Read the model definition and answer for the solid it produces. Units are mm, in the model's axes. A direction names the side the tool comes from. Coordinates: 2 decimals unless noted, no trailing zeros. Loops run counter-clockwise (first coordinate to the right, second up) from the corner with the lowest first, then second, coordinate; pieces in that order, holes last. Notation, with made-up numbers: (52, 28) - (79, 28) arc R15 cw to (79, 42) - close; hole circle Ø9 at (69.5, 36.5). An arc over 180 degrees is marked (long way). One line per item, written item: value. Start each with the question number.
from build123d import *

# Parameters (mm, degrees)
SKETCH_1_R          = 5.25
EXTRUDE_1_DEPTH     = 10
EXTRUDE_2_DEPTH     = 30
SKETCH_3_R          = 10
CUT_EXTRUDE_1_DEPTH = 134
FILLET_1_R          = 5


with BuildPart() as part:
    # 草图1 → 凸台-拉伸1 (new body)
    with BuildSketch(Plane.XY):
        with BuildLine():
            Line((-120, -130), (120, -130))
            ThreePointArc((120, -130), (127.071067812, -127.071067812), (130, -120))
            Line((130, -120), (130, 120))
            ThreePointArc((130, 120), (127.071067812, 127.071067812), (120, 130))
            Line((120, 130), (-120, 130))
            ThreePointArc((-120, 130), (-127.071067812, 127.071067812), (-130, 120))
            Line((-130, 120), (-130, -120))
            ThreePointArc((-130, -120), (-127.071067812, -127.071067812), (-120, -130))
        make_face()
        with Locations((-115, 115)):
            Circle(SKETCH_1_R, mode=Mode.SUBTRACT)
        with Locations((115, 115)):
            Circle(SKETCH_1_R, mode=Mode.SUBTRACT)
        with Locations((115, -115)):
            Circle(SKETCH_1_R, mode=Mode.SUBTRACT)
        with Locations((-115, -115)):
            Circle(SKETCH_1_R, mode=Mode.SUBTRACT)
    extrude(amount=EXTRUDE_1_DEPTH)

    # 草图2 → 凸台-拉伸2 (add, symmetric)
    with BuildSketch(Plane(origin=(0, 0, 0), x_dir=(1, 0, 0), z_dir=(0, 1, 0))):
        with BuildLine():
            Line((-50, -10), (50, -10))
            Line((50, -10), (20, -27.278852826))
            Line((20, -27.278852826), (20, -55))
            ThreePointArc((20, -55), (0, -75), (-20, -55))
            Line((-20, -55), (-20, -27.278852826))
            Line((-20, -27.278852826), (-50, -10))
        make_face()
    extrude(amount=EXTRUDE_2_DEPTH, both=True)

    # 草图3 → 切除-拉伸1 (cut)
    with BuildSketch(Plane.XZ.offset(30)):
        with Locations(Location((0, 55, 0), (0, 0, 270))):
            Circle(SKETCH_3_R)
    extrude(amount=-CUT_EXTRUDE_1_DEPTH, mode=Mode.SUBTRACT)

    # 圆角1
    fillet_1_edges = [part.edges().sort_by_distance(p)[0] for p in [
        (-20, 0, 27.278852826),
        (20, 0, 27.278852826),
    ]]
    fillet(fillet_1_edges, radius=FILLET_1_R)


solid = part.part
1) Section D-D, the plane y = 11.5 is taken. Determine the outline of the cut face in (x, z).
2) Section B-B, the plane y = 115 is taken. Determine the outline of the cut face in (x, z).
3) Section A-A, the plane x = 0 is taken. Determine the outline of the cut face in (y, z), and give its area (3 significant figures).
4) Flat-ended cylindrical pins translate along their axes: P1, Ø10, axis at x = -84.5, y = 35, coming from the +Z side; P2, Ø1.5, axis at x = -33.5, z = 19.5, coming from the -Y side; P3, Ø20, axis at y = 11.5, z = 36.5, coming from the -X side. Find the tip coordinate at first contact, or state that the pin passes through.
5) For faces 1 (the flat face through (1, 30, 35)), 2 (the flat face through (-20, 0, 43)), 3 (the flat face through (36.44, 0.42, 17.81)), determine the directions among +Z, -Z, +X, -X, +Y, -Y from which every point of the face is accessible in a straight line to the end or side of a thin tool.
6) Determine the mould class of faces 4 (the flat face through (20, 0, 42)), 5 (the cylindrical face through (-110, -113.4, 4.9)), 6 (the cylindrical face through (-127.15, -126.99, 4.93)) for opening direction Y: released by +Y, released by -Y, zero draft, split by the parting line, or undercut.
7) Straight lines are drawn through the part: L1, parallel to Y at x = 115, z = 4; L2, parallel to Z at x = -24.5, y = 45; L3, parallel to X at y = 5, z = 52. For each, find the intervals that lie inside material, in ascending order.
Answer below:
1. outline: (-130, 0) - (130, 0) - (130, 10) - (50, 10) - (22.5, 25.84) arc R5 cw to (20, 30.17) - (20, 55) arc R20 ccw to (-20, 55) - (-20, 30.17) arc R5 cw to (-22.5, 25.84) - (-50, 10) - (-130, 10) - close; hole circle Ø20 at (0, 55)
2. outline: (-130, 0) - (-120.25, 0) - (-120.25, 10) - (-130, 10) - close; (-109.75, 0) - (109.75, 0) - (109.75, 10) - (-109.75, 10) - close; (120.25, 0) - (130, 0) - (130, 10) - (120.25, 10) - close
3. outline: (-130, 0) - (130, 0) - (130, 10) - (30, 10) - (30, 45) - (-30, 45) - (-30, 10) - (-130, 10) - close; (-30, 65) - (30, 65) - (30, 75) - (-30, 75) - close
3. area: 5,300 mm2
4. P1: z = 10
4. P2: y = -30
4. P3: x = -21.6
5. face 1: +Z, +X, -X, +Y
5. face 2: +Z, -X, +Y, -Y
5. face 3: +Z, +X, +Y, -Y
6. face 4: zero draft
6. face 5: undercut
6. face 6: released by -Y
7. L1: -130 to -120.25, -109.75 to 109.75, 120.25 to 130
7. L2: 0 to 10
7. L3: -20 to -9.54, 9.54 to 20
